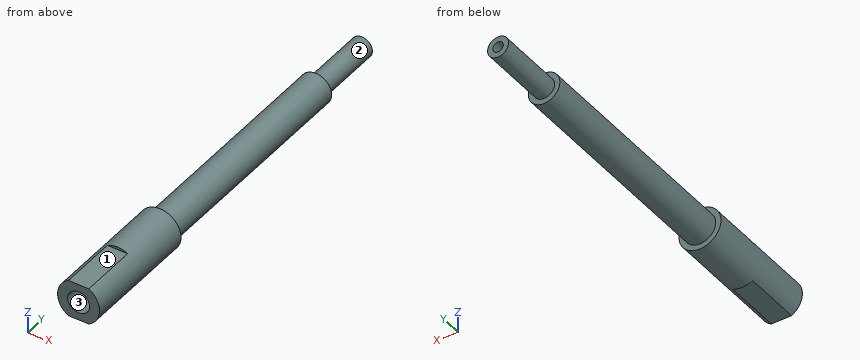
```python
from build123d import *

# Parameters (mm, degrees)
SKETCH5_R                  = 1
CUT_EXTRUDE2_DEPTH         = 81.199750623
M5X0_75_TAPPED_HOLE1_D     = 4.2
M5X0_75_TAPPED_HOLE1_DEPTH = 12.25
M5X0_75_TAPPED_HOLE1_TIP   = 1.2618073
CUT_EXTRUDE3_DEPTH         = 81.199750623
CUT_EXTRUDE3_DEPTH_BACK    = 81.199750623
SKETCH6_W                  = 4.168944331
SKETCH6_H                  = 22.175025747
SKETCH6_W_2                = 2.42822795
SKETCH7_R                  = 3
BOSS_EXTRUDE1_DEPTH        = 5


with BuildPart() as part:
    # Sketch1 → Revolve1 (revolve)
    with BuildSketch(Plane.XY, mode=Mode.PRIVATE) as revolve1_sk:
        Polygon((3, 23), (4, 23), (4, 0), (0, 0), (0, 80), (2, 80), (2, 62), (3, 62), align=None)
    revolve(revolve1_sk.sketch.rotate(Axis((0, 80, 0), (0, -1, 0)), 180), axis=Axis((0, 80, 0), (0, -1, 0)))

    # Sketch5 → Cut-Extrude2 (cut, through all)
    with BuildSketch(Plane(origin=(0, 80, 0), x_dir=(1, 0, 0), z_dir=(0, 1, 0))):
        with Locations(Location((0, 0, 0), (0, 0, 180))):
            Circle(SKETCH5_R)
    extrude(amount=-CUT_EXTRUDE2_DEPTH, mode=Mode.SUBTRACT)

    # M5x0.75 Tapped Hole1
    with Locations(Plane(origin=(0, 0, 0), x_dir=(-1, 0, 0), z_dir=(0, -1, 0))):
        with Locations((0, 0)):
            Hole(M5X0_75_TAPPED_HOLE1_D / 2, depth=M5X0_75_TAPPED_HOLE1_DEPTH)
            with Locations((0, 0, -(M5X0_75_TAPPED_HOLE1_DEPTH + M5X0_75_TAPPED_HOLE1_TIP / 2))):  # 118° drill point
                Cone(0, M5X0_75_TAPPED_HOLE1_D / 2, M5X0_75_TAPPED_HOLE1_TIP, mode=Mode.SUBTRACT)

    # Sketch6 → Cut-Extrude3 (cut, two sides: drawn at the far end of the back side and taken through both)
    with BuildSketch(Plane(origin=(0, 0, 0), x_dir=(0, 0, -1), z_dir=(1, 0, 0)).offset(-CUT_EXTRUDE3_DEPTH_BACK)):
        with Locations((-5.584472166, -0.087512874)):
            Rectangle(SKETCH6_W, SKETCH6_H)
        with Locations((4.714113975, -0.087512874)):
            Rectangle(SKETCH6_W_2, SKETCH6_H)
    extrude(amount=CUT_EXTRUDE3_DEPTH + CUT_EXTRUDE3_DEPTH_BACK, mode=Mode.SUBTRACT)

    # Sketch7 → Boss-Extrude1 (add)
    with BuildSketch(Plane(origin=(0, 62, 0), x_dir=(1, 0, 0), z_dir=(0, 1, 0))):
        with Locations(Location((0, 0, 0), (0, 0, 180))):
            Circle(SKETCH7_R)
    extrude(amount=BOSS_EXTRUDE1_DEPTH)


solid = part.part
```
Source: CAD feature listing. Evaluate the final solid. Frame: model axes, mm. Face numbers are marked on the shaded views. A direction names the side the tool comes from. Round coordinates to 2 decimals unless told otherwise and drop trailing zeros. Loops run counter-clockwise (first coordinate to the right, second up) from the corner with the lowest first, then second, coordinate; pieces in that order, holes last.
1. Section query C-C on y = 14. Output: boundary loops of the cut face in (x, z).
2. Contact query for flat-ended pins moving along their axis: pin 1 (1.6 mm diameter, centred on x = 0, z = 0.5, fed in from -Y); pin 2 (0.6 mm diameter, centred on x = 0.5, z = -4, fed in from -Y); pin 3 (1.6 mm diameter, centred on x = 0, z = 0, fed in from +Y); pin 4 (4 mm diameter, centred on y = 18, z = -1, fed in from -X). Output: stop coordinate, or through.
3. Ray query, L1, parallel to Z at x = 0, y = 70; L2, parallel to Z at x = 0, y = 5; L3, parallel to X at y = 44.5, z = 0. Return the intervals inside material, ascending.
4. Section query D-D on y = 51. Output: boundary loops of the cut face in (x, z), and give its area (3 significant figures).
5. Section query B-B on x = 0. Output: boundary loops of the cut face in (y, z), and give its area (3 significant figures).
6. Section query A-A on z = 0. Output: boundary loops of the cut face in (x, y), and give its area (3 significant figures).
7. Access query for the marked faces 1, 2 and 3. Directions: +Z, -Z, +X, -X, +Y, -Y. A direction counts if a zero-diameter tool reaches every point of the face in a straight line with its end or side. Return the directions, or none.
Answers below:
1. outline: circle Ø8 at (0, 0); hole circle Ø2 at (0, 0)
2. pin 1: stops at y = 12.73
2. pin 2: stops at y = 11
2. pin 3: stops at y = 67
2. pin 4: stops at x = -4
3. L1: z = -2 to -1, 1 to 2
3. L2: z = -3.5 to -2.1, 2.1 to 3.5
3. L3: x = -3 to -1, 1 to 3
4. outline: circle Ø6 at (0, 0); hole circle Ø2 at (0, 0)
4. area: 25.1 mm2
5. outline: (0, -3.5) - (11, -3.5) - (11, -4) - (23, -4) - (23, -3) - (67, -3) - (67, -2) - (80, -2) - (80, -1) - (67, -1) - (67, 1) - (80, 1) - (80, 2) - (67, 2) - (67, 3) - (23, 3) - (23, 4) - (11, 4) - (11, 3.5) - (0, 3.5) - (0, 2.1) - (12.25, 2.1) - (12.91, 1) - (62, 1) - (62, -1) - (12.91, -1) - (12.25, -2.1) - (0, -2.1) - close
5. area: 311 mm2
6. outline: (-4, 0) - (-2.1, 0) - (-2.1, 12.25) - (-1, 12.91) - (-1, 62) - (1, 62) - (1, 12.91) - (2.1, 12.25) - (2.1, 0) - (4, 0) - (4, 23) - (3, 23) - (3, 67) - (2, 67) - (2, 80) - (1, 80) - (1, 67) - (-1, 67) - (-1, 80) - (-2, 80) - (-2, 67) - (-3, 67) - (-3, 23) - (-4, 23) - close
6. area: 322 mm2
7. face 1: +Z, +X, -X, -Y
7. face 2: +Y
7. face 3: -Y
